Design review of the part built by this model. Coordinates are the model's own, in mm. A direction names the side the tool comes from. Give positions to 0.01 mm unless a question says otherwise; leave off trailing zeros. Loops run counter-clockwise (first coordinate to the right, second up) from the corner with the lowest first, then second, coordinate; pieces in that order, holes last. Notation, with made-up numbers: (9, -22) - (31, -22) arc R25 ccw to (31, -6) - close; hole circle Ø10 at (-9.75, -35). An arc over 180 degrees is marked (long way). Write each question's results on one line, items separated by ' | '.
```python
from build123d import *

# Parameters (mm, degrees)
SKETCH1_R           = 6
BOSS_EXTRUDE1_DEPTH = 15
SKETCH2_R           = 8
BOSS_EXTRUDE2_DEPTH = 30
BOSS_EXTRUDE3_START = 15
SKETCH3_R           = 6
BOSS_EXTRUDE3_DEPTH = 15
CHAMFER1_SIZE       = 0.5


with BuildPart() as part:
    # Sketch1 → Boss-Extrude1 (new body)
    with BuildSketch(Plane.XY):
        Circle(SKETCH1_R)
    extrude(amount=BOSS_EXTRUDE1_DEPTH)

    # Sketch2 → Boss-Extrude2 (add)
    with BuildSketch(Plane(origin=(0, 0, 0), x_dir=(-1, 0, 0), z_dir=(0, 0, -1))):
        Circle(SKETCH2_R)
    extrude(amount=BOSS_EXTRUDE2_DEPTH)

    # Sketch3 → Boss-Extrude3 (add)
    with BuildSketch(Plane(origin=(0, 0, -30), x_dir=(-1, 0, 0), z_dir=(0, 0, -1)).offset(BOSS_EXTRUDE3_START)):
        with Locations(Location((0, 0, 0), (0, 0, 180))):
            Circle(SKETCH3_R)
    extrude(amount=-BOSS_EXTRUDE3_DEPTH)

    # Chamfer1
    chamfer1_edges = [part.edges().sort_by_distance(p)[0] for p in [
        (-6, 0, -45),
        (-6, 0, 15),
        (8, 0, 0),
        (8, 0, -30),
    ]]
    chamfer(chamfer1_edges, length=CHAMFER1_SIZE)


solid = part.part
```
Item 1: Tool access review of faces 1 (the face through (-6, 0, 7)), 2 (the face through (0, 0, 15)), 3 (the face through (5.723, -1.802, -37.352)): name each direction out of +Z, -Z, +X, -X, +Y, -Y from which nothing blocks a thin tool from reaching the whole face with its end or side.
Output values:
face 1: +Z | face 2: +Z, +X, -X, +Y, -Y | face 3: -Z
Item 2: We need section C-C on z = -38.5. Give the boundary of the cut face in (x, y), then the cut area to 3 significant figures.
Output values:
outline: circle Ø12 at (0, 0) | area: 113 mm²
Item 3: We need section A-A on y = 0. Give the boundary of the cut face in (x, z).
Output values:
outline: (-8, -29.5) - (-7.5, -30) - (-6, -30) - (-6, -44.5) - (-5.5, -45) - (5.5, -45) - (6, -44.5) - (6, -30) - (7.5, -30) - (8, -29.5) - (8, -0.5) - (7.5, 0) - (6, 0) - (6, 14.5) - (5.5, 15) - (-5.5, 15) - (-6, 14.5) - (-6, 0) - (-7.5, 0) - (-8, -0.5) - close
Item 4: We need section D-D on z = -26. Give the boundary of the cut face in (x, y), then the cut area to 3 significant figures.
Output values:
outline: circle Ø16 at (0, 0) | area: 201 mm²
Item 5: Wall thickness on probe 1 along X at (y, z) = (-0.25, -19); probe 2 along Z at (x, y) = (-0.5, 7); probe 3 along Y at (x, z) = (0.25, -39): over which ranges is each line inside the solid? List them lowest first.
Output values:
probe 1: x = -8 to 8 | probe 2: z = -30 to 0 | probe 3: y = -5.99 to 5.99
